CAD build for the part. Positions are in the model's coordinates, mm. A direction names the side the tool comes from. Round coordinates to 2 decimals unless told otherwise and drop trailing zeros. Order: outer loops, then holes, each group sorted by start corner. A loop starts at its lowest first (then second) coordinate and runs counter-clockwise, first axis right, second up. Notation, with made-up numbers: M -23,-33.5 L 14,-33.5 A18 ccw 14,-10.5 Z; hole C 86,2 d2. An arc over 180 degrees is marked long. Answer as a JSON object with one key per item and string values.
```python
from build123d import *

# Parameters (mm, degrees)
EXTRUDE_1_DEPTH     = 100
CUT_EXTRUDE_1_DEPTH = 100
SKETCH_3_R          = 6.5
CUT_EXTRUDE_2_DEPTH = 100
FILLET_1_R          = 10


with BuildPart() as part:
    # 草图1 → 凸台-拉伸1 (new body)
    with BuildSketch(Plane.XY):
        Polygon((0, 0), (-100, 0), (-100, -75), (-92, -75), (-92, -8), (0, -8), align=None)
    extrude(amount=EXTRUDE_1_DEPTH)

    # 草图2 → 切除-拉伸1 (cut)
    with BuildSketch(Plane(origin=(0, 0, 0), x_dir=(1, 0, 0), z_dir=(0, 1, 0))):
        with BuildLine():
            Line((-38.5, -13.5), (-21.5, -13.5))
            ThreePointArc((-21.5, -13.5), (-15, -20), (-21.5, -26.5))
            Line((-21.5, -26.5), (-38.5, -26.5))
            ThreePointArc((-38.5, -26.5), (-45, -20), (-38.5, -13.5))
        make_face()
        with BuildLine():
            Line((-38.5, -73.5), (-21.5, -73.5))
            ThreePointArc((-21.5, -73.5), (-15, -80), (-21.5, -86.5))
            Line((-21.5, -86.5), (-38.5, -86.5))
            ThreePointArc((-38.5, -86.5), (-45, -80), (-38.5, -73.5))
        make_face()
    extrude(amount=-CUT_EXTRUDE_1_DEPTH, mode=Mode.SUBTRACT)

    # 草图3 → 切除-拉伸2 (cut)
    with BuildSketch(Plane(origin=(-92, 0, 0), x_dir=(0, 0, -1), z_dir=(1, 0, 0))):
        with Locations((-80, -45)):
            Circle(SKETCH_3_R)
        with Locations((-20, -45)):
            Circle(SKETCH_3_R)
    extrude(amount=-CUT_EXTRUDE_2_DEPTH, mode=Mode.SUBTRACT)

    # 圆角1
    fillet_1_edges = [part.edges().sort_by_distance(p)[0] for p in [
        (-92, -8, 50),
    ]]
    fillet(fillet_1_edges, radius=FILLET_1_R)


solid = part.part
```
Item 1: Drop a flat-ended pin along its axis: pin 1 Ø3 at (y, z) = (-61, 87.5) entering from +X. Give the stop position or say it passes through.
Worked answers:
{"pin 1": "stops at x = -92"}
Item 2: 3-axis set-ups, long thin cutter, end or side, ignore diameter. For faces 1 (the flat face through (-42, -8, 49)), 2 (the flat face through (-30, -4, 86.5)), 3 (the cylindrical face through (-95.9, -47.5, 74)): which of +Z, -Z, +X, -X, +Y, -Y reach the whole face in a straight line?
Worked answers:
{"face 1": "+Z, -Z, +X, -Y", "face 2": "+Y, -Y", "face 3": "+X, -X"}
Item 3: Saw through at C-C on z = 8. List the corners of the cut face in (x, y).
Worked answers:
{"outline": "M -100,-75 L -92,-75 L -92,-18 A10 cw -82,-8 L 0,-8 L 0,0 L -100,0 Z"}
Item 4: Saw through at A-A on y = -45. List the corners of the cut face in (x, z).
Worked answers:
{"outline": "M -100,0 L -92,0 L -92,13.5 L -100,13.5 Z; M -100,26.5 L -92,26.5 L -92,73.5 L -100,73.5 Z; M -100,86.5 L -92,86.5 L -92,100 L -100,100 Z"}
Item 5: Saw through at B-B on z = 80. List the corners of the cut face in (x, y).
Worked answers:
{"outline": "M -100,-75 L -92,-75 L -92,-51.5 L -100,-51.5 Z; M -100,-38.5 L -92,-38.5 L -92,-18 A10 cw -82,-8 L -45,-8 L -45,0 L -100,0 Z; M -15,-8 L 0,-8 L 0,0 L -15,0 Z"}
Item 6: Saw through at D-D on y = -25.5. List the corners of the cut face in (x, z).
Worked answers:
{"outline": "M -100,0 L -92,0 L -92,100 L -100,100 Z"}
Item 7: Wall check: line 1 along Y through (x, z) = (-96, 80); line 2 along Y through (x, z) = (-55, 73.5); line 3 along X through (y, z) = (-39.5, 93). Give the ranges that are in metal, low to high. Write a range as [from, to].
Worked answers:
{"line 1": "y = [-75, -51.5], [-38.5, 0]", "line 2": "y = [-8, 0]", "line 3": "x = [-100, -92]"}
Item 8: Two-plate mould, pull along X, no slides. Class faces 4 (the flat face through (-100, -37, 49)), 5 (the flat face through (-69, -7, 100)), 6 (the flat face through (-30, -4, 13.5)), 7 (the flat face through (0, -4, 49)): released by +X, released by -X, zero draft, split by the parting line, or undercut.
Worked answers:
{"face 4": "released by -X", "face 5": "zero draft", "face 6": "undercut", "face 7": "released by +X"}
